```python
from build123d import *

# Parameters (mm, degrees)
SKETCH1_W           = 1000
SKETCH1_H           = 530
BOSS_EXTRUDE1_DEPTH = 350
FILLET1_R           = 5
SKETCH3_W           = 5
SKETCH3_H           = 530
CUT_EXTRUDE2_DEPTH  = 2
CUT_EXTRUDE3_DEPTH  = 5
SKETCH5_W           = 450
SKETCH5_H           = 60
CUT_EXTRUDE4_DEPTH  = 1
FILLET2_R           = 10


with BuildPart() as part:
    # Sketch1 → Boss-Extrude1 (new body)
    with BuildSketch(Plane.XY):
        Rectangle(SKETCH1_W, SKETCH1_H)
    extrude(amount=BOSS_EXTRUDE1_DEPTH)

    # Fillet1
    fillet1_edges = [part.edges().sort_by_distance(p)[0] for p in [
        (-500, 0, 350),
        (0, -265, 350),
        (500, 0, 350),
        (0, -265, 0),
        (-500, 0, 0),
        (0, 265, 0),
        (500, 0, 0),
        (0, 265, 350),
        (500, -265, 175),
        (-500, -265, 175),
        (-500, 265, 175),
        (500, 265, 175),
    ]]
    fillet(fillet1_edges, radius=FILLET1_R)

    # Sketch3 → Cut-Extrude2 (cut)
    with BuildSketch(Plane.XY.offset(350)):
        Rectangle(SKETCH3_W, SKETCH3_H)
    extrude(amount=-CUT_EXTRUDE2_DEPTH, mode=Mode.SUBTRACT)

    # Sketch4 → Cut-Extrude3 (cut)
    with BuildSketch(Plane.XY.offset(350)):
        with BuildLine():
            Line((65, 60), (65, -60))
            ThreePointArc((65, -60), (50, -75), (35, -60))
            Line((35, -60), (35, 60))
            ThreePointArc((35, 60), (50, 75), (65, 60))
        make_face()
    extrude(amount=-CUT_EXTRUDE3_DEPTH, mode=Mode.SUBTRACT)

    # Sketch5 → Cut-Extrude4 (cut)
    with BuildSketch(Plane.XZ.offset(265)):
        with Locations((0, 175)):
            Rectangle(SKETCH5_W, SKETCH5_H)
    extrude(amount=-CUT_EXTRUDE4_DEPTH, mode=Mode.SUBTRACT)

    # Fillet2
    fillet2_edges = [part.edges().sort_by_distance(p)[0] for p in [
        (225, -264.5, 205),
        (225, -264.5, 145),
        (-225, -264.5, 145),
        (-225, -264.5, 205),
    ]]
    fillet(fillet2_edges, radius=FILLET2_R)


solid = part.part
```
Check sheet for the modelled part. Datum: model origin and axes. Units: mm. A direction names the side the tool comes from. Coordinates: 2 decimals unless noted, no trailing zeros. Write each question's results on one line, items separated by ' | '. Start each with the question number.
1. Access from +Z, -Z, +X, -X, +Y, -Y to the whole of each face (thin tool, end or side, straight path). Record for faces 4 (the face through (50, 1, 345)), 5 (the face through (-252, 4, 350)).
2. Material ranges on probe 1 along Y at (x, z) = (115, 182.5), recorded low to high.
3. Go/stop test with flat-tipped pins: P1, Ø1.1, axis at x = -43.5, y = -264.5, coming from the -Z side; P2, Ø15, axis at x = 56.5, y = -36, coming from the +Z side; P3, Ø1.1, axis at y = -264.5, z = 183.5, coming from the -X side. Record where each tip stops, or that it passes through.
4. Mould release check, pull along Z, two halves, no side actions. Record for faces 1 (the face through (-7, -265, 135)), 2 (the face through (245, 4, 350)), 3 (the face through (-3, -264, 175)): +Z half, -Z half, draft (parallel to the pull), parting line (faces both ways), or undercut.
Checks:
1) face 4: +Z | face 5: +Z, +X, -X, +Y, -Y
2) probe 1: y = -264 to 265
3) P1: stops at z = 1.93 | P2: stops at z = 345 | P3: stops at x = -498.07
4) face 1: draft | face 2: +Z half | face 3: undercut
